Source: CAD feature listing. Evaluate the final solid. Frame: model axes, mm. A direction names the side the tool comes from. Give positions to 0.01 mm unless a question says otherwise; leave off trailing zeros. Write each loop counter-clockwise with the first axis right and the second up, starting at its lowest first coordinate (ties: lowest second). Pieces come first, ordered by that corner, then holes. Notation, with made-up numbers: M 54,-7.5 L 60,-7.5 A15 cw 60,14.5 Z; hole C 10,-36.5 d10. An arc over 180 degrees is marked long. Return JSON: item names as keys, results as strings.
```python
from build123d import *

# Parameters (mm, degrees)
EXTRUDE_THIN1_DEPTH = 4
CUT_EXTRUDE1_DEPTH  = 28.129319933
CUT_EXTRUDE2_DEPTH  = 29.017851452
FILLET1_R           = 1


with BuildPart() as part:
    # Sketch1 → Extrude-Thin1 (new, symmetric)
    with BuildSketch(Plane.XY):
        Polygon((12, 0), (0, 0), (0, 25), (1, 25), (1, 1), (12, 1), align=None)
    extrude(amount=EXTRUDE_THIN1_DEPTH, both=True)

    # Sketch2 → Cut-Extrude1 (cut, through all)
    with BuildSketch(Plane(origin=(0, 1, 0), x_dir=(1, 0, 0), z_dir=(0, 1, 0))):
        with BuildLine():
            Line((6, 1.75), (9, 1.75))
            ThreePointArc((9, 1.75), (10.75, 0), (9, -1.75))
            Line((9, -1.75), (6, -1.75))
            ThreePointArc((6, -1.75), (4.25, 0), (6, 1.75))
        make_face()
    extrude(amount=-CUT_EXTRUDE1_DEPTH, mode=Mode.SUBTRACT)

    # Sketch3 → Cut-Extrude2 (cut, through all)
    with BuildSketch(Plane.ZY):
        with BuildLine():
            Line((-1.75, 16), (-1.75, 21))
            ThreePointArc((-1.75, 21), (0, 22.75), (1.75, 21))
            Line((1.75, 21), (1.75, 16))
            ThreePointArc((1.75, 16), (0, 14.25), (-1.75, 16))
        make_face()
    extrude(amount=-CUT_EXTRUDE2_DEPTH, mode=Mode.SUBTRACT)

    # Fillet1
    fillet1_edges = [part.edges().sort_by_distance(p)[0] for p in [
        (0.5, 25, 4),
        (0.5, 25, -4),
        (12, 0.5, -4),
        (12, 0.5, 4),
        (0, 0, 0),
        (1, 1, 0),
    ]]
    fillet(fillet1_edges, radius=FILLET1_R)


solid = part.part
```
1) Set-up query: faces 4 (the face through (1, 14, 0)), 5 (the face through (0.6, 8.5, 4)), 6 (the face through (0.507, 24.699, -3.715)), 7 (the face through (7.5, 0.5, 1.75)), 8 (the face through (0.5, 18.5, -1.75)). Return all of +Z, -Z, +X, -X, +Y, -Y with unobstructed straight access to the full face (end or side cutting, diameter ignored); none if empty.
Numbers:
{"face 4": "+Z, -Z, +X, +Y", "face 5": "+Z, +X, -X, +Y, -Y", "face 6": "-Z, +X, -X, +Y", "face 7": "+Y, -Y", "face 8": "+X, -X"}
2) Line query: line 1 (X direction, y = 10.25, z = -0.5); line 2 (Y direction, x = 1.5, z = 2.25). Output: solid intervals per line, ascending. Write a range as [from, to].
Numbers:
{"line 1": "x = [0, 1]", "line 2": "y = [0, 1.13]"}
3) Cut plane C-C, the plane z = 0. Return the cut outline in (x, y).
Numbers:
{"outline": "M 0,1 A1 ccw 1,0 L 4.25,0 L 4.25,1 L 2,1 A1 cw 1,2 L 1,14.25 L 0,14.25 Z; M 0,22.75 L 1,22.75 L 1,25 L 0,25 Z; M 10.75,0 L 12,0 L 12,1 L 10.75,1 Z"}
4) Cut plane D-D, the plane x = 3.5. Return the cut outline in (y, z).
Numbers:
{"outline": "M 0,-4 L 1,-4 L 1,4 L 0,4 Z"}
5) Draft query along X for faces 1 (the face through (0, 13, 0)), 2 (the face through (12, 0.5, 0)), 3 (the face through (4.25, 0.51, 0.04)). Return one class per face: released by +X, released by -X, zero draft, split by the parting line, or undercut.
Numbers:
{"face 1": "released by -X", "face 2": "released by +X", "face 3": "undercut"}
6) Cut plane A-A, the plane x = 7.5. Return the cut outline in (y, z), then the cut area to 3 significant figures.
Numbers:
{"outline": "M 0,-4 L 1,-4 L 1,-1.75 L 0,-1.75 Z; M 0,1.75 L 1,1.75 L 1,4 L 0,4 Z", "area": "4.50 mm²"}
7) Contact query for flat-ended pins moving along their axis: pin 1 Ø4 at (y, z) = (8.5, 2) entering from +X; pin 2 Ø4 at (x, z) = (8, -1) entering from +Y. Output: stop coordinate, or through.
Numbers:
{"pin 1": "stops at x = 1", "pin 2": "stops at y = 1"}
